Drawing for the job (mm, zero at the part's lowest x, y, z). A direction names the side the tool comes from. Round coordinates to 2 decimals unless told otherwise and drop trailing zeros. Write each loop counter-clockwise with the first axis right and the second up, starting at its lowest first coordinate (ties: lowest second). Pieces come first, ordered by that corner, then holes. Notation, with made-up numbers: (61, 58) - (84, 58) arc R13 ccw to (84, 67) - close; hole circle Ø9 at (-2, -34.5). An arc over 180 degrees is marked (long way). Answer in a Markdown table with one row per item.
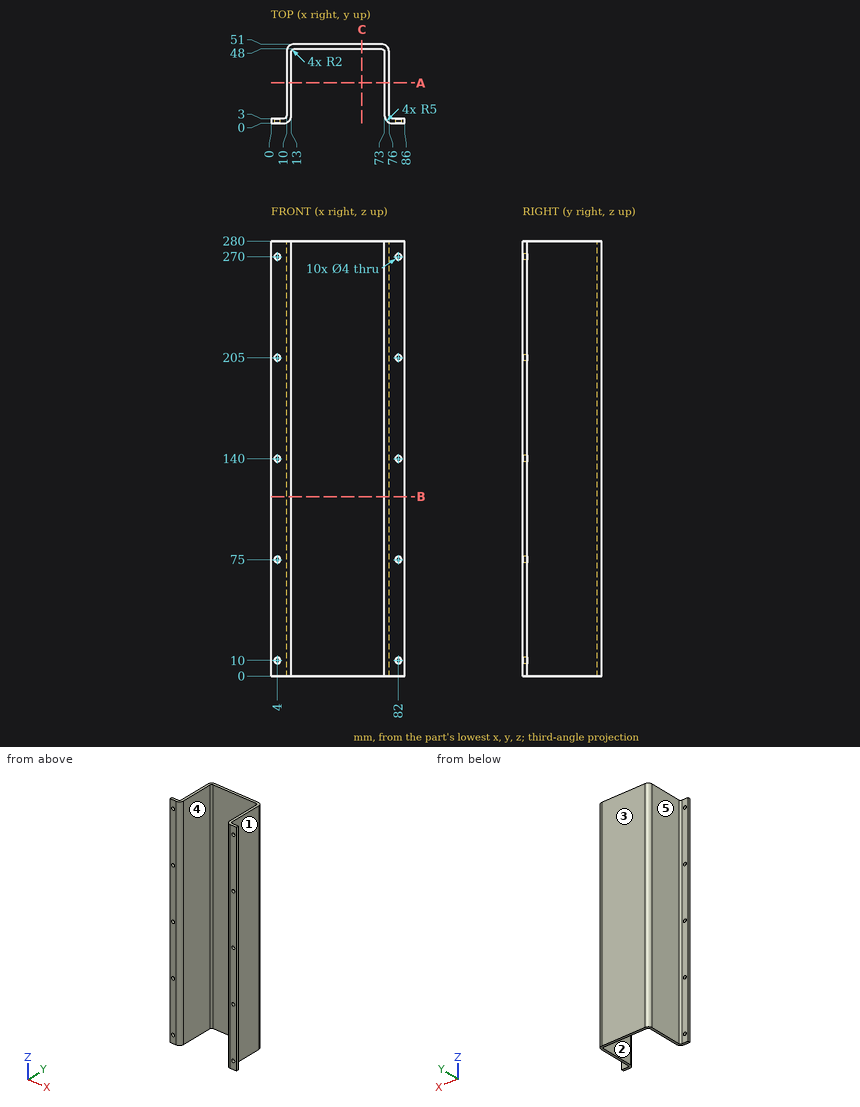
Q1. Saw through at C-C on x = 58.5. List the corners of the cut face in (y, z).
Computed:
| item | result |
|---|---|
| outline | (48, 0) - (51, 0) - (51, 280) - (48, 280) - close |
Q2. Flat gauge pins, fed straight in: pin 1 (4.5 mm diameter, centred on x = 4, z = 140, fed in from +Y); pin 2 (20.5 mm diameter, centred on y = 31.5, z = 111, fed in from +X); pin 3 (8 mm diameter, centred on y = 22, z = 191.5, fed in from -X). Where does each tip first touch, or does it go through?
Computed:
| item | result |
|---|---|
| pin 1 | stops at y = 3 |
| pin 2 | stops at x = 76 |
| pin 3 | stops at x = 10 |
Q3. Saw through at A-A on y = 26. List the corners of the cut face in (x, z).
Computed:
| item | result |
|---|---|
| outline | (10, 0) - (13, 0) - (13, 280) - (10, 280) - close; (73, 0) - (76, 0) - (76, 280) - (73, 280) - close |
Q4. Saw through at B-B on z = 115.5. List the corners of the cut face in (x, y).
Computed:
| item | result |
|---|---|
| outline | (0, 0) - (8, 0) arc R5 ccw to (13, 5) - (13, 46) arc R2 cw to (15, 48) - (71, 48) arc R2 cw to (73, 46) - (73, 5) arc R5 ccw to (78, 0) - (86, 0) - (86, 3) - (78, 3) arc R2 cw to (76, 5) - (76, 46) arc R5 ccw to (71, 51) - (15, 51) arc R5 ccw to (10, 46) - (10, 5) arc R2 cw to (8, 3) - (0, 3) - close |
Q5. 3-axis set-ups, long thin cutter, end or side, ignore diameter. For the marked faces 1 and 2: which of +Z, -Z, +X, -X, +Y, -Y reach the whole face in a straight line?
Computed:
| item | result |
|---|---|
| face 1 | +Z, -Z, +X, +Y |
| face 2 | +Z, -Z, -Y |
Q6. Pull direction X, two halves, no side cores. Call the marked faces 3, 4 and 5: released by +X, released by -X, zero draft, split by the parting line, or undercut.
Computed:
| item | result |
|---|---|
| face 3 | zero draft |
| face 4 | undercut |
| face 5 | released by -X |
Q7. Drill centre lines: line 1 (Z direction, x = 82, y = 0.6); line 2 (X direction, y = 1.25, z = 270); line 3 (X direction, y = 38, z = 144). Where is each one in solid material? Low to high.
Computed:
| item | result |
|---|---|
| line 1 | z = 0 to 8, 12 to 73, 77 to 138, 142 to 203, 207 to 268, 272 to 280 |
| line 2 | x = 0 to 2, 6 to 11.31, 74.69 to 80, 84 to 86 |
| line 3 | x = 10 to 13, 73 to 76 |
